Verification items for this drawing (mm, ordinates from the low corner). Coordinates: 2 decimals unless noted, no trailing zeros. Write each loop counter-clockwise with the first axis right and the second up, starting at its lowest first coordinate (ties: lowest second). Pieces come first, ordered by that corner, then holes.
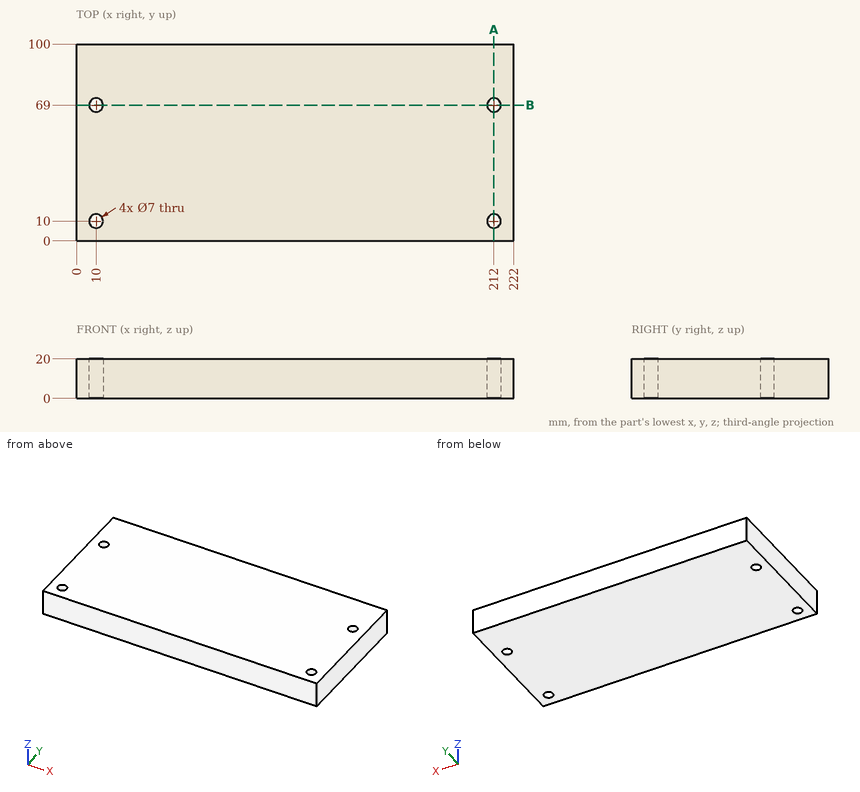
1. Thickness scan on line 1 along Y through (x, z) = (212, 15.25); line 2 along X through (y, z) = (66.5, 12.5); line 3 along X through (y, z) = (11, 16.75). Record the ranges inside material, lowest first.
Computed values:
line 1: y = 0 to 6.5, 13.5 to 65.5, 72.5 to 100
line 2: x = 0 to 7.55, 12.45 to 209.55, 214.45 to 222
line 3: x = 0 to 6.65, 13.35 to 208.65, 215.35 to 222
2. Sectioned sample at A-A, the plane x = 212. Record the boundary of the cut face in (y, z).
Computed values:
outline: (0, 0) - (6.5, 0) - (6.5, 20) - (0, 20) - close; (13.5, 0) - (65.5, 0) - (65.5, 20) - (13.5, 20) - close; (72.5, 0) - (100, 0) - (100, 20) - (72.5, 20) - close
3. Sectioned sample at B-B, the plane y = 69. Record the boundary of the cut face in (x, z), and give its area (3 significant figures).
Computed values:
outline: (0, 0) - (6.5, 0) - (6.5, 20) - (0, 20) - close; (13.5, 0) - (208.5, 0) - (208.5, 20) - (13.5, 20) - close; (215.5, 0) - (222, 0) - (222, 20) - (215.5, 20) - close
area: 4,160 mm2
4. Gauge pin test, flat end, axial feed: pin 1 Ø4 at (x, y) = (10, 69) entering from -Z. Record the tip position at first contact, or that the pin passes through.
Computed values:
pin 1: passes through
